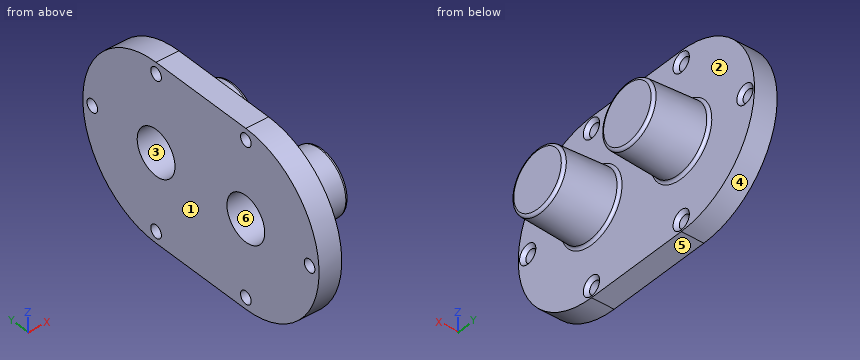
```python
from build123d import *

# Parameters (mm, degrees)
BOSS_EXTRUDE1_DEPTH            = 8
F_16_0_16_DIAMETER_HOLE1_D     = 16
F_16_0_16_DIAMETER_HOLE1_DEPTH = 24
F_4_5_4_5_DIAMETER_HOLE1_D     = 4.5
CHAMFER1_SIZE                  = 1.2
FILLET1_R                      = 1


with BuildPart() as part:
    # Sketch1 → Boss-Extrude1 (new body)
    with BuildSketch(Plane(origin=(8, 0, 0), x_dir=(0, 0, -1), z_dir=(1, 0, 0))):
        with BuildLine():
            Line((31, -19), (31, 19))
            ThreePointArc((31, 19), (0, 50), (-31, 19))
            Line((-31, 19), (-31, -19))
            ThreePointArc((-31, -19), (0, -50), (31, -19))
        make_face()
    extrude(amount=-BOSS_EXTRUDE1_DEPTH)

    # Sketch2 → Revolve1 (revolve)
    with BuildSketch(Plane.XY, mode=Mode.PRIVATE) as revolve1_sk:
        Polygon((8, -7.004252194), (8, -19), (27, -19), (27, -8), align=None)
    revolve(revolve1_sk.sketch.rotate(Axis((8, -19, 0), (1, 0, 0)), 270), axis=Axis((8, -19, 0), (1, 0, 0)))

    # Sketch3 → Revolve2 (revolve)
    with BuildSketch(Plane.XY, mode=Mode.PRIVATE) as revolve2_sk:
        Polygon((8, 30.995747806), (8, 19), (27, 19), (27, 30), align=None)
    revolve(revolve2_sk.sketch.rotate(Axis((8, 19, 0), (1, 0, 0)), 270), axis=Axis((8, 19, 0), (1, 0, 0)))

    # Ø16.0 (16) Diameter Hole1
    with Locations(Plane.ZY):
        with Locations((0, 19), (0, -19)):
            Hole(F_16_0_16_DIAMETER_HOLE1_D / 2, depth=F_16_0_16_DIAMETER_HOLE1_DEPTH)

    # Ø4.5 (4.5) Diameter Hole1 (through all)
    with Locations(Plane(origin=(8, 0, 0), x_dir=(0, 0, -1), z_dir=(1, 0, 0))):
        with Locations((0, 46), (-27, 19), (27, 19), (-27, -19), (27, -19), (0, -46)):
            Hole(F_4_5_4_5_DIAMETER_HOLE1_D / 2)

    # Chamfer1
    chamfer1_edges = [part.edges().sort_by_distance(p)[0] for p in [
        (8, -46, -2.25),
        (8, -19, -29.25),
        (8, -19, 24.75),
        (8, 19, -29.25),
        (8, 19, 24.75),
        (8, 46, -2.25),
    ]]
    chamfer(chamfer1_edges, length=CHAMFER1_SIZE)

    # Fillet1
    fillet1_edges = [part.edges().sort_by_distance(p)[0] for p in [
        (8, -19, 11.995747806),
        (27, -19, 11),
        (8, 19, 11.995747806),
        (27, 19, 11),
    ]]
    fillet(fillet1_edges, radius=FILLET1_R)


solid = part.part
```
Read the model definition and answer for the solid it produces. Units are mm, in the model's axes. Face numbers are marked on the shaded views. A direction names the side the tool comes from. Give positions to 0.01 mm unless a question says otherwise; leave off trailing zeros. Write each loop counter-clockwise with the first axis right and the second up, starting at its lowest first coordinate (ties: lowest second). Pieces come first, ordered by that corner, then holes. Notation, with made-up numbers: (7, 65) - (53, 65) arc R38 cw to (53, 104) - close; hole circle Ø10 at (-35.5, 86). An arc over 180 degrees is marked (long way). Write item = value, one per line. Start each with the question number.
Item 1: A tool of negligible diameter and unlimited length cuts with its end or side. For the marked faces 1, 2 and 3, from which of +Z, -Z, +X, -X, +Y, -Y can it reach the whole face along a straight path? Write none if from no direction.
Item 2: Find section A-A (x = 4). State how many separate pieces and enclosed holes the cut face has, then the cut area to 3 significant figures.
Item 3: The mould has two halves that part along Y. Classify the marked faces 4, 5 and 6: +Y half, -Y half, draft (parallel to the pull), parting line (faces both ways), or undercut.
Item 4: Find section B-B (z = -27). Give the vertices of the cut face in (x, y).
Item 5: Find section C-C (y = -46). Give the vertices of the cut face in (x, z).
Item 6: Find the intervals of material crossed by probe 1 along Y at (x, z) = (4.5, 27); probe 2 along X at (y, z) = (-2.5, -28); probe 3 along Z at (x, y) = (5.75, -21), in increasing order. Write a range as [from, to].
Item 7: Find section D-D (x = 18). Give the vertices of the cut face in (y, z).
Item 8: Each of these flat-tipped pins is pushed along its axis until it touches: P1, Ø2.5, axis at y = -46, z = 0, coming from the -X side; P2, Ø10, axis at x = 12.5, z = -18, coming from the +Y side; P3, Ø6, axis at x = 12.5, z = 6.5, coming from the +Y side; P4, Ø5, axis at x = 21.5, z = 12, coming from the -Y side. Where does it stop, or does it pass through?
Response:
q1.face_1 = +Z, -Z, -X, +Y, -Y
q1.face_2 = +X
q1.face_3 = -X
q2.separate_pieces = 1
q2.enclosed_holes = 8
q2.area = 4,880 mm²
q3.face_4 = +Y half
q3.face_5 = draft
q3.face_6 = undercut
q4.outline = (0, -34.23) - (8, -34.23) - (8, -22.45) - (6.8, -21.25) - (0, -21.25) - close; (0, -16.75) - (6.8, -16.75) - (8, -15.55) - (8, 15.55) - (6.8, 16.75) - (0, 16.75) - close; (0, 21.25) - (6.8, 21.25) - (8, 22.45) - (8, 34.23) - (0, 34.23) - close
q5.outline = (0, -15.23) - (8, -15.23) - (8, -3.45) - (6.8, -2.25) - (0, -2.25) - close; (0, 2.25) - (6.8, 2.25) - (8, 3.45) - (8, 15.23) - (0, 15.23) - close
q6.probe_1 = [-34.23, -21.25], [-16.75, 16.75], [21.25, 34.23]
q6.probe_2 = [0, 8]
q6.probe_3 = [-30.94, -28.03], [-25.97, -7.75], [7.75, 25.97], [28.03, 30.94]
q7.outline = circle Ø22.94 at (-19, 0); circle Ø22.94 at (19, 0); hole circle Ø16 at (-19, 0); hole circle Ø16 at (19, 0)
q8.P1 = through
q8.P2 = 45.66
q8.P3 = 30.24
q8.P4 = -25.1
